Verification items for the finished model (mm, model axes). A direction names the side the tool comes from. Coordinates: 2 decimals unless noted, no trailing zeros. Write each loop counter-clockwise with the first axis right and the second up, starting at its lowest first coordinate (ties: lowest second). Pieces come first, ordered by that corner, then holes. Notation, with made-up numbers: (3, -35) -> (26, -35) arc R15 ccw to (26, -28) -> close; hole circle Ø3 at (-10.5, 43.5). An arc over 180 degrees is marked (long way). Answer in a Markdown table with one row per item.
```python
from build123d import *

# Parameters (mm, degrees)
EXTRUDE_1_DEPTH     = 4
SKETCH_3_R          = 6.4
EXTRUDE_2_DEPTH     = 8
CUT_EXTRUDE_1_REACH = 34.792
SKETCH_4_R          = 3
CHAMFER_1_SIZE      = 0.5


with BuildPart() as part:
    # 草图1 → 旋转1 (revolve)
    with BuildSketch(Plane.XY, mode=Mode.PRIVATE) as revolve_1_sk:
        Polygon((-5, 4), (-4.5, 7), (-5, 7), (-5, 8), (-4.5, 11), (-5, 11), (-5, 12), (-4.5, 15), (-5, 15), (-5, 16), (-4.5, 19), (0, 19), (0, 0), (-5, 0), align=None)
    revolve(revolve_1_sk.sketch.rotate(Axis((0, 0, 0), (0, 1, 0)), 270), axis=Axis((0, 0, 0), (0, 1, 0)))

    # 草图2 → 凸台-拉伸1 (add)
    with BuildSketch(Plane.XZ):
        Polygon((8.082903769, 0), (4.041451884, 7), (-4.041451884, 7), (-8.082903769, 0), (-4.041451884, -7), (4.041451884, -7), align=None)
    extrude(amount=EXTRUDE_1_DEPTH)

    # 草图3 → 凸台-拉伸2 (add)
    with BuildSketch(Plane.XZ.offset(4)):
        Circle(SKETCH_3_R)
    extrude(amount=EXTRUDE_2_DEPTH)

    # 草图4 → 切除-拉伸1 (cut, up to next)
    with BuildSketch(Plane(origin=(0, 19, 0), x_dir=(1, 0, 0), z_dir=(0, 1, 0)), mode=Mode.PRIVATE) as cut_extrude_1_sk1:
        with Locations(Location((0, 0, 0), (0, 0, 180))):
            Circle(SKETCH_4_R)
    cut_extrude_1_tool1 = extrude(cut_extrude_1_sk1.sketch, amount=-CUT_EXTRUDE_1_REACH, mode=Mode.PRIVATE) & part.part
    add(cut_extrude_1_tool1.solids().sort_by_distance((0, 19, 0))[0], mode=Mode.SUBTRACT)

    # 倒角1
    chamfer_1_edges = [part.edges().sort_by_distance(p)[0] for p in [
        (-6.4, -12, 0),
    ]]
    chamfer(chamfer_1_edges, length=CHAMFER_1_SIZE)


solid = part.part
```
1. Go/stop test with flat-tipped pins: pin 1 (6 mm diameter, centred on y = 8.5, z = 1, fed in from -X); pin 2 (5 mm diameter, centred on x = -5.5, y = 15, fed in from +Z). Record where each tip stops, or that it passes through.
Findings below:
| item | result |
|---|---|
| pin 1 | stops at x = -5 |
| pin 2 | stops at z = 4 |
2. Sectioned sample at A-A, the plane y = 3. Record the cut outline in (x, z).
Findings below:
| item | result |
|---|---|
| outline | circle Ø10 at (0, 0); hole circle Ø6 at (0, 0) |
3. Sectioned sample at B-B, the plane y = 16.5. Record the cut outline in (x, z).
Findings below:
| item | result |
|---|---|
| outline | circle Ø9.83 at (0, 0); hole circle Ø6 at (0, 0) |
4. Material ranges on probe 1 along Z at (x, y) = (0, -4.5); probe 2 along X at (y, z) = (0.5, 1.25); probe 3 along Z at (x, y) = (-2, 6), recorded low to high. Write a range as from..to.
Findings below:
| item | result |
|---|---|
| probe 1 | z = -6.4..-3, 3..6.4 |
| probe 2 | x = -4.84..-2.73, 2.73..4.84 |
| probe 3 | z = -4.22..-2.24, 2.24..4.22 |
5. Access from +Z, -Z, +X, -X, +Y, -Y to the whole of each face (thin tool, end or side, straight path). Record for faces 1 (the face through (3, -4, 6)), 2 (the face through (6.034, -1.972, -3.549)), 3 (the face through (-1.39, 6.19, -4.42)), 4 (the face through (4.88, 2.03, 1.08)).
Findings below:
| item | result |
|---|---|
| face 1 | -Y |
| face 2 | -Z, +X, +Y, -Y |
| face 3 | none |
| face 4 | +Y |
6. Release check for a two-part mould opening along X. For faces 5 (the face through (0, -2, 7)), 6 (the face through (-6.09, -1.97, -3.45)), 7 (the face through (-2.86, 3.72, 0.9)) record: released by +X, released by -X, zero draft, split by the parting line, or undercut.
Findings below:
| item | result |
|---|---|
| face 5 | zero draft |
| face 6 | released by -X |
| face 7 | undercut |
